from build123d import *

# Parameters (mm, degrees)
SKETCH1_R              = 20
SKETCH1_R_2            = 12.5
BOSS_EXTRUDE1_DEPTH    = 10
CUT_EXTRUDE1_DEPTH     = 31
M5_TAPPED_HOLE1_REACH  = 46.091
M5_TAPPED_HOLE1_BORE_R = 2.1
M3_TAPPED_HOLE1_D      = 2.5


with BuildPart() as part:
    # Sketch1 → Boss-Extrude1 (new body)
    with BuildSketch(Plane(origin=(0, 0, 0), x_dir=(1, 0, 0), z_dir=(0, 1, 0))):
        with Locations(Location((0, 0, 0), (0, 0, 270))):
            Circle(SKETCH1_R)
        with Locations(Location((0, 0, 0), (0, 0, 270))):
            Circle(SKETCH1_R_2, mode=Mode.SUBTRACT)
    extrude(amount=BOSS_EXTRUDE1_DEPTH)

    # Sketch2 → Cut-Extrude1 (cut, through all)
    with BuildSketch(Plane(origin=(0, 10, 0), x_dir=(1, 0, 0), z_dir=(0, 1, 0))):
        with BuildLine():
            Line((8.717797887, 18), (-8.717797887, 18))
            ThreePointArc((-8.717797887, 18), (0, 20), (8.717797887, 18))
        make_face()
    extrude(amount=-CUT_EXTRUDE1_DEPTH, mode=Mode.SUBTRACT)

    # M5 Tapped Hole1 bore → M5 Tapped Hole1 (cut, up to next)
    with BuildSketch(Plane(origin=(0, 0, -18), x_dir=(-1, 0, 0), z_dir=(0, 0, -1)), mode=Mode.PRIVATE) as m5_tapped_hole1_sk1:
        with Locations((0, 5)):
            Circle(M5_TAPPED_HOLE1_BORE_R)
    m5_tapped_hole1_tool1 = extrude(m5_tapped_hole1_sk1.sketch, amount=-M5_TAPPED_HOLE1_REACH, mode=Mode.PRIVATE) & part.part
    add(m5_tapped_hole1_tool1.solids().sort_by_distance((0, 5, -18))[0], mode=Mode.SUBTRACT)

    # M3 Tapped Hole1 (through all)
    with Locations(Plane(origin=(0, 0, 0), x_dir=(-1, 0, 0), z_dir=(0, -1, 0))):
        with Locations((-11.490485194, 11.490485194), (11.490485194, 11.490485194), (-11.490485194, -11.490485194), (11.490485194, -11.490485194)):
            Hole(M3_TAPPED_HOLE1_D / 2)


solid = part.part
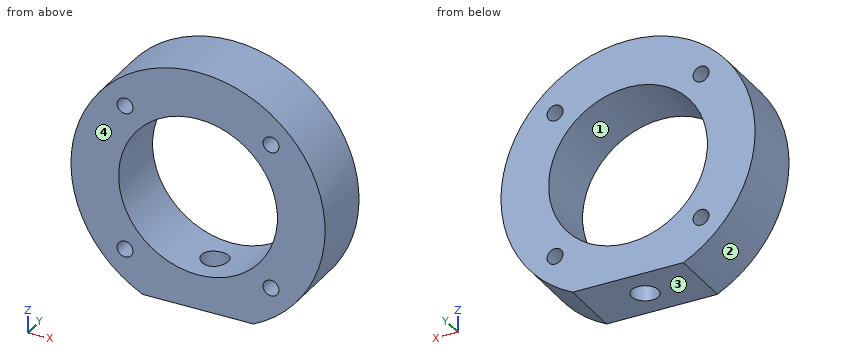
Build history of the part. All positions in model axes, mm. Face numbers are marked on the shaded views. Round coordinates to 2 decimals unless told otherwise and drop trailing zeros. Write each loop counter-clockwise with the first axis right and the second up, starting at its lowest first coordinate (ties: lowest second). Pieces come first, ordered by that corner, then holes. Notation, with made-up numbers: (64.25, 75) - (100.25, 75) arc R13 ccw to (100.25, 82) - close; hole circle Ø1 at (52.25, -5). An arc over 180 degrees is marked (long way). Use CSV: the item, a comma, the result in double quotes.
(1) Pin check, flat tips, straight feed: P1, Ø1.5, axis at x = 2, y = 1.5, coming from the +Z side; P2, Ø2, axis at y = 6.5, z = 7, coming from the -X side; P3, Ø4, axis at y = 7.5, z = 16, coming from the -X side. Stop position of each tip, or through.
Response:
P1,"z = 19.96"
P2,"x = -19.08"
P3,"x = -14.28"
(2) Band-saw the part on D-D (y = 5). Write the cut outline in (x, z).
Response:
outline,"(-8.72, -18) - (-2.1, -18) - (-2.1, -12.32) arc R12.5 cw (long way) to (2.1, -12.32) - (2.1, -18) - (8.72, -18) arc R20 ccw (long way) to start; hole circle Ø2.5 at (-11.49, -11.49); hole circle Ø2.5 at (-11.49, 11.49); hole circle Ø2.5 at (11.49, -11.49); hole circle Ø2.5 at (11.49, 11.49)"
(3) Band-saw the part on C-C (x = 4). Write the cut outline in (y, z).
Response:
outline,"(0, -18) - (10, -18) - (10, -11.84) - (0, -11.84) - close; (0, 11.84) - (10, 11.84) - (10, 19.6) - (0, 19.6) - close"
(4) Band-saw the part on B-B (z = 0). Write the cut outline in (x, y).
Response:
outline,"(-20, 0) - (-12.5, 0) - (-12.5, 10) - (-20, 10) - close; (12.5, 0) - (20, 0) - (20, 10) - (12.5, 10) - close"
(5) Wall check: line 1 (X direction, y = 4.5, z = 8); line 2 (Z direction, x = -6, y = 8.5); line 3 (Z direction, x = 6.5, y = 7.75). Give the ranges that are in metal, low to high.
Response:
line 1,"-18.33 to -9.6, 9.6 to 18.33"
line 2,"-18 to -10.97, 10.97 to 19.08"
line 3,"-18 to -10.68, 10.68 to 18.91"
(6) Band-saw the part on A-A (x = 0). Write the cut outline in (y, z).
Response:
outline,"(0, -18) - (2.9, -18) - (2.9, -12.5) - (0, -12.5) - close; (0, 12.5) - (10, 12.5) - (10, 20) - (0, 20) - close; (7.1, -18) - (10, -18) - (10, -12.5) - (7.1, -12.5) - close"
(7) Mould opens along Z. For the marked faces 1, 2, 3 and 4 say: pulls with the +Z half, pulls with the -Z half, needs draft (parallel to the pull), parting line crosses it, or undercut.
Response:
face 1,"undercut"
face 2,"parting line crosses it"
face 3,"pulls with the -Z half"
face 4,"needs draft"
